```python
from build123d import *

# Parameters (mm, degrees)
SKETCH_4_W             = 1
SKETCH_4_H             = 1.2
CUT_EXTRUDE_1_DEPTH    = 50
PATTERN_LINEAR_1_COUNT = 10
PATTERN_LINEAR_1_PITCH = 0.7


with BuildPart() as part:
    # 草图3 → Revolve 915 (revolve)
    with BuildSketch(Plane.XY, mode=Mode.PRIVATE) as revolve_915_sk:
        with BuildLine():
            Line((0, 0), (10.4, 0))
            Line((10.4, 0), (10.4, 2))
            Line((10.4, 2), (3.8, 2))
            Line((3.8, 2), (3.532, 1.732))
            Line((3.532, 1.732), (3.018, 1.732))
            ThreePointArc((3.018, 1.732), (2.581008009, 1.913008009), (2.4, 2.35))
            Line((2.4, 2.35), (2.4, 4))
            Line((2.4, 4), (1.095413109, 3.885863436))
            ThreePointArc((1.095413109, 3.885863436), (0.315267196, 3.501138048), (0, 2.690429799))
            Line((0, 2.690429799), (0, 0))
        make_face()
    revolve(revolve_915_sk.sketch.rotate(Axis((-2.477021524, 0, 0), (1, 0, 0)), 90), axis=Axis((-2.477021524, 0, 0), (1, 0, 0)))

    # 草图4 → 切除-拉伸1 (cut, symmetric)
    with BuildSketch(Plane.XY):
        with Locations((0.5, 0)):
            Rectangle(SKETCH_4_W, SKETCH_4_H)
    extrude(amount=CUT_EXTRUDE_1_DEPTH, both=True, mode=Mode.SUBTRACT)

    # 草图5 → 切除-旋转1 (revolve, cut)
    with BuildSketch(Plane.XY, mode=Mode.PRIVATE) as cut_revolve_1_sk:
        Polygon((10.046208796, 2), (10.746208796, 2), (10.4, 1.3938), align=None)
    cut_revolve_1 = revolve(cut_revolve_1_sk.sketch.rotate(Axis((6.174994867, 0, 0), (-1, 0, 0)), 270), axis=Axis((6.174994867, 0, 0), (-1, 0, 0)), mode=Mode.SUBTRACT)

    # 阵列(线性)1: 切除-旋转1 ×10
    with Locations(*[(-i * PATTERN_LINEAR_1_PITCH, 0, 0) for i in range(1, PATTERN_LINEAR_1_COUNT)]):
        add(cut_revolve_1, mode=Mode.SUBTRACT)


solid = part.part
```
Could you check a few things on this model? Use its own coordinates, in mm. A direction names the side the tool comes from. Round coordinates to 2 decimals unless told otherwise and drop trailing zeros. One line per question, with ' | ' between items.
Q1. Which directions (+Z, -Z, +X, -X, +Y, -Y) give clear straight access to the entire face, cutting with the end or side of a thin tool? Please do faces 1 (the face through (10.4, 0, 0)), 2 (the face through (2.4, 2, -2)), 3 (the face through (0.5, -0.6, 0.1)).
Computed values:
face 1: +Z, -Z, +X, +Y, -Y | face 2: +X | face 3: +Z, -Z, -X
Q2. I'm going to push flat-ended pins straight in: pin 1 (3 mm diameter, centred on x = 7.5, z = 0.5, fed in from -Y); pin 2 (1.1 mm diameter, centred on x = 0.5, z = 1, fed in from -Y); pin 3 (0.5 mm diameter, centred on x = 0.5, z = 0, fed in from +Y). Where does each tip first touch, or does it pass through?
Computed values:
pin 1: y = -2 | pin 2: y = -3.8 | pin 3: y = 3.8
Q3. If I drill on line 1 (X direction, y = -2, z = 1.5); line 2 (Y direction, x = 2.5, z = -0.25), over which ranges is the centre line in solid material (lowest first)? Write a range as from..to.
Computed values:
line 1: 0..2.4 | line 2: -2..2
Q4. We'd pull the mould along Y, two halves only. Please class faces 4 (the face through (0, 1, 0)), 5 (the face through (1, 0, 0)): released by +Y, released by -Y, zero draft, split by the parting line, or undercut.
Computed values:
face 4: zero draft | face 5: undercut
